Input: part model. Units: mm. Frame: model coordinates. Coordinates: 2 decimals unless noted, no trailing zeros. Loops run counter-clockwise (first coordinate to the right, second up) from the corner with the lowest first, then second, coordinate; pieces in that order, holes last.
```python
from build123d import *

# Parameters (mm, degrees)
SKETCH_1_W      = 95
SKETCH_1_H      = 380
SKETCH_1_R      = 6.5
EXTRUDE_2_DEPTH = 4


with BuildPart() as part:
    # 草图1 → 凸台-拉伸2 (new body)
    with BuildSketch(Plane.XY):
        with Locations((47.5, -190)):
            Rectangle(SKETCH_1_W, SKETCH_1_H)
        with Locations((15, -302.5)):
            Circle(SKETCH_1_R, mode=Mode.SUBTRACT)
        with Locations((15, -222.5)):
            Circle(SKETCH_1_R, mode=Mode.SUBTRACT)
    extrude(amount=EXTRUDE_2_DEPTH)


solid = part.part
```
Item 1: Line query: L1, parallel to Y at x = 15, z = 0.8; L2, parallel to Y at x = 12, z = 2.8; L3, parallel to X at y = -302.5, z = 1.35. Output: solid intervals per line, ascending.
Result:
L1: y = -380 to -309, -296 to -229, -216 to 0
L2: y = -380 to -308.27, -296.73 to -228.27, -216.73 to 0
L3: x = 0 to 8.5, 21.5 to 95
Item 2: Section query B-B (x = 15). Output: boundary loops of the cut face in (y, z), then the cut area to 3 significant figures.
Result:
outline: (-380, 0) - (-309, 0) - (-309, 4) - (-380, 4) - close; (-296, 0) - (-229, 0) - (-229, 4) - (-296, 4) - close; (-216, 0) - (0, 0) - (0, 4) - (-216, 4) - close
area: 1,420 mm2
Item 3: Section query A-A (y = -222.5). Output: boundary loops of the cut face in (x, z), then the cut area to 3 significant figures.
Result:
outline: (0, 0) - (8.5, 0) - (8.5, 4) - (0, 4) - close; (21.5, 0) - (95, 0) - (95, 4) - (21.5, 4) - close
area: 328 mm2
Item 4: Mould query, pull axis X, two halves, no side actions, for faces 1 (the face through (18.494, -297.019, 1.972)), 2 (the face through (47, -187, 4)). Classes: +X half, -X half, draft (parallel to the pull), parting line (faces both ways), or undercut.
Result:
face 1: undercut
face 2: draft
Item 5: Contact query for a flat-ended pin moving along its axis: P1, Ø11.5, axis at x = 15, y = -222.5, coming from the -Z side. Output: stop coordinate, or through.
Result:
P1: passes through
